Verification items for the finished model (mm, model axes). Give positions to 0.01 mm unless a question says otherwise; leave off trailing zeros. Loops run counter-clockwise (first coordinate to the right, second up) from the corner with the lowest first, then second, coordinate; pieces in that order, holes last. Notation, with made-up numbers: (-30, -10.75) - (-10, -10.75) arc R31 cw to (-10, 15.25) - close; hole circle Ø3 at (62.5, -34). An arc over 180 degrees is marked (long way). One line per item, written item: value. Start each with the question number.
1. Sectioned sample at B-B (y = 13.5). Record the cut outline in (x, z).
2. Sectioned sample at A-A (z = -17). Record the cut outline in (x, y).
3. Sectioned sample at C-C (y = -16). Record the cut outline in (x, z).
4. Scan lines: L1, parallel to X at y = 14.5, z = -73; L2, parallel to X at y = 15.5, z = 62.5; L3, parallel to Y at x = 17, z = 13.5. Record each from-to range of solid material in increasing order. Write a range as [from, to].
5. Gauge pin test, flat ends, axial feed: pin 1 (3 mm diameter, centred on y = 17, z = 24.5, fed in from +X); pin 2 (1.5 mm diameter, centred on y = -11, z = -80.5, fed in from +X); pin 3 (6 mm diameter, centred on y = -14.5, z = -80.5, fed in from +X). Record the tip position at first contact, or that the pin passes through.
from build123d import *

# Parameters (mm, degrees)
SKETCH1_W           = 250
SKETCH1_H           = 50
BOSS_EXTRUDE1_DEPTH = 25
CHAMFER1_SIZE       = 20


with BuildPart() as part:
    # Sketch1 → Boss-Extrude1 (new, symmetric)
    with BuildSketch(Plane(origin=(0, 0, 0), x_dir=(0, 0, -1), z_dir=(1, 0, 0))):
        Rectangle(SKETCH1_W, SKETCH1_H)
    extrude(amount=BOSS_EXTRUDE1_DEPTH, both=True)

    # Chamfer1
    chamfer1_edges = [part.edges().sort_by_distance(p)[0] for p in [
        (25, 25, 0),
        (25, -25, 0),
    ]]
    chamfer(chamfer1_edges, length=CHAMFER1_SIZE)


solid = part.part
Results are:
1. outline: (-25, -125) - (16.5, -125) - (16.5, 125) - (-25, 125) - close
2. outline: (-25, -25) - (5, -25) - (25, -5) - (25, 5) - (5, 25) - (-25, 25) - close
3. outline: (-25, -125) - (14, -125) - (14, 125) - (-25, 125) - close
4. L1: x = [-25, 15.5]
4. L2: x = [-25, 14.5]
4. L3: y = [-13, 13]
5. pin 1: stops at x = 14.5
5. pin 2: stops at x = 19.75
5. pin 3: stops at x = 18.5
